Geometry: final body of the model. Coordinates: model frame, mm. A direction names the side the tool comes from. Give positions to 0.01 mm unless a question says otherwise; leave off trailing zeros. Write each loop counter-clockwise with the first axis right and the second up, starting at its lowest first coordinate (ties: lowest second). Pieces come first, ordered by that corner, then holes.
Q1. Reachability of faces 1 (the face through (28, 1, -50)), 2 (the face through (-12, 44, 31)), 3 (the face through (8, -1, -62.5)), 4 (the face through (-14, -22, 1)) from +Z, -Z, +X, -X, +Y, -Y: full face, straight path, thin tool, end or side. Return the list, or none.
Q2. Cut plane D-D on z = -58. Return the cut outline in (x, y), plus the area to 3 significant figures.
Q3. Cut plane B-B on y = -5. Return the cut outline in (x, z).
Q4. Draft query along X for faces 5 (the face through (0.816, 63.72, -19.983)), 6 (the face through (-8, -27, 1)), 7 (the face through (20, -1, 1)), 8 (the face through (0, -44, 1)). Return one class per face: pulls with the +X half, pulls with the -X half, needs draft (parallel to the pull), parting line crosses it, or undercut.
Q5. Pin query (flat end, axial travel): pin 1 (12.5 mm diameter, centred on x = 13, z = 29, fed in from +Y); pin 2 (4 mm diameter, centred on x = 7, y = 42, fed in from -Z); pin 3 (13 mm diameter, centred on x = -13, z = 12, fed in from -Y); pin 4 (11 mm diameter, centred on y = -25, z = -1.5, fed in from +X). Return the tip coordinate at first contact, or that it passes through.
Q6. Cut plane A-A on z = -75. Return the cut outline in (x, y).
Q7. Line query: L1, parallel to Z at x = 17.5, y = -39; L2, parallel to Y at x = -7, z = 20.5; L3, parallel to X at y = 62, z = 0. Output: solid intervals per line, ascending.
Q8. Cut plane C-C on x = 0. Return the cut outline in (y, z), plus the area to 3 significant figures.
```python
from build123d import *

# Parameters (mm, degrees)
BASE_BLOCK_SKETCH_W         = 40
BASE_BLOCK_SKETCH_H         = 88
BASE_BLOCK_DEPTH            = 50
C_CHANNEL_CUT_DEPTH         = 112.067547015
SLOTTED_LUG_DEPTH           = 40
LUG_START                   = 16
LUG_RIM_DEPTH               = 16
BOSS_CYLINDER_SKETCH_18_R   = 20
BOSS_CYLINDER_SKETCH_18_R_2 = 9
BOSS_CYLINDER_18_DEPTH      = 40
BOSS_EXTENSION_DEPTH        = 40
BOSS_BORE_CUT_DEPTH         = 40
GUSSET_RIB_A_SKETCH_W       = 40
GUSSET_RIB_A_SKETCH_H       = 4
GUSSET_RIB_A_DEPTH          = 10
GUSSET_RIB_B_SKETCH_W       = 40
GUSSET_RIB_B_SKETCH_H       = 4
GUSSET_RIB_B_DEPTH          = 10


with BuildPart() as part:
    # Base Block Sketch → Base Block (new, symmetric)
    with BuildSketch(Plane.XY):
        Rectangle(BASE_BLOCK_SKETCH_W, BASE_BLOCK_SKETCH_H)
    extrude(amount=BASE_BLOCK_DEPTH, both=True)

    # C-Channel Cut Sketch → C-Channel Cut (cut, through all)
    with BuildSketch(Plane.XY.offset(50)):
        Polygon((-20, 22), (-8, 22), (-8, 32), (8, 32), (8, -32), (-8, -32), (-8, -22), (-20, -22), align=None)
    extrude(amount=-C_CHANNEL_CUT_DEPTH, mode=Mode.SUBTRACT)

    # Slotted Lug Sketch → Slotted Lug (add, through all)
    with BuildSketch(Plane(origin=(20, 0, 0), x_dir=(0, 0, -1), z_dir=(1, 0, 0))):
        with BuildLine():
            Line((100, -40), (100, 40))
            ThreePointArc((100, 40), (75, 65), (50, 40))
            Line((50, 40), (50, -40))
            ThreePointArc((50, -40), (75, -65), (100, -40))
        make_face()
        with BuildLine():
            Line((62.5, -40), (62.5, 40))
            ThreePointArc((62.5, 40), (75, 52.5), (87.5, 40))
            Line((87.5, 40), (87.5, -40))
            ThreePointArc((87.5, -40), (75, -52.5), (62.5, -40))
        make_face(mode=Mode.SUBTRACT)
    extrude(amount=-SLOTTED_LUG_DEPTH)

    # Lug Rim Sketch → Lug Rim (add)
    with BuildSketch(Plane(origin=(20, 0, 0), x_dir=(0, 0, -1), z_dir=(1, 0, 0)).offset(LUG_START)):
        with BuildLine():
            Line((50, 40), (50, -40))
            ThreePointArc((50, -40), (75, -65), (100, -40))
            Line((100, -40), (100, 40))
            ThreePointArc((100, 40), (75, 65), (50, 40))
        make_face()
        with BuildLine():
            ThreePointArc((62.5, 40), (75, 52.5), (87.5, 40))
            Line((87.5, 40), (87.5, -40))
            ThreePointArc((87.5, -40), (75, -52.5), (62.5, -40))
            Line((62.5, -40), (62.5, 40))
        make_face(mode=Mode.SUBTRACT)
    extrude(amount=-LUG_RIM_DEPTH)

    # Boss Cylinder Sketch Ø18 → Boss Cylinder Ø18 (add)
    with BuildSketch(Plane(origin=(0, 44, 0), x_dir=(1, 0, 0), z_dir=(0, 1, 0))):
        with Locations(Location((0, 0, 0), (0, 0, 180))):
            Circle(BOSS_CYLINDER_SKETCH_18_R)
        with Locations(Location((0, 0, 0), (0, 0, 270))):
            Circle(BOSS_CYLINDER_SKETCH_18_R_2, mode=Mode.SUBTRACT)
    extrude(amount=BOSS_CYLINDER_18_DEPTH)

    # Boss Extension Sketch → Boss Extension (add)
    with BuildSketch(Plane(origin=(0, 44, 0), x_dir=(1, 0, 0), z_dir=(0, 1, 0))):
        with BuildLine():
            Line((-4.5, -19.48717527), (-4.5, -50))
            Line((-4.5, -50), (4.5, -50))
            Line((4.5, -50), (4.5, -19.48717527))
            ThreePointArc((4.5, -19.48717527), (0, -20), (-4.5, -19.48717527))
        make_face()
    extrude(amount=BOSS_EXTENSION_DEPTH)

    # Boss Bore Sketch → Boss Bore Cut (cut)
    with BuildSketch(Plane.ZY.offset(4.5)):
        Polygon((19.48717527, 84), (50, 44), (50, 84), align=None)
    extrude(amount=-BOSS_BORE_CUT_DEPTH, mode=Mode.SUBTRACT)

    # Gusset Rib A Sketch → Gusset Rib A (add)
    with BuildSketch(Plane(origin=(0, 0, -50), x_dir=(-1, 0, 0), z_dir=(0, 0, -1))):
        with Locations((0, 42)):
            Rectangle(GUSSET_RIB_A_SKETCH_W, GUSSET_RIB_A_SKETCH_H)
    extrude(amount=GUSSET_RIB_A_DEPTH)

    # Gusset Rib B Sketch → Gusset Rib B (add)
    with BuildSketch(Plane(origin=(0, 0, -50), x_dir=(-1, 0, 0), z_dir=(0, 0, -1))):
        with Locations((0, -42)):
            Rectangle(GUSSET_RIB_B_SKETCH_W, GUSSET_RIB_B_SKETCH_H)
    extrude(amount=GUSSET_RIB_B_DEPTH)


solid = part.part
```
Data:
1. face 1: +Z, +X, +Y, -Y
1. face 2: +Z, -X, +Y
1. face 3: +X, -X
1. face 4: +Z, -X
2. outline: (-20, -58.33) - (36, -58.33) - (36, 58.33) - (-20, 58.33) - close
2. area: 6,530 mm2
3. outline: (-20, -100) - (36, -100) - (36, -87.5) - (-20, -87.5) - close; (-20, -62.5) - (36, -62.5) - (36, -50) - (20, -50) - (20, 50) - (8, 50) - (8, -50) - (-20, -50) - close
4. face 5: parting line crosses it
4. face 6: undercut
4. face 7: pulls with the +X half
4. face 8: needs draft
5. pin 1: stops at y = 44
5. pin 2: stops at z = -100
5. pin 3: stops at y = -44
5. pin 4: stops at x = 20
6. outline: (-20, -65) - (36, -65) - (36, -52.5) - (-20, -52.5) - close; (-20, 52.5) - (36, 52.5) - (36, 65) - (-20, 65) - close
7. L1: z = -100 to -87.5, -62.5 to 50
7. L2: y = -44 to -32, 32 to 44
7. L3: x = -20 to -9, 9 to 20
8. outline: (-44, -50.32) arc R25 ccw to (-40, -100) - (40, -100) arc R25 ccw to (44, -50.32) - (44, -20) - (84, -20) - (84, -9) - (44, -9) - (44, 9) - (84, 9) - (84, 19.49) - (44, 50) - (32, 50) - (32, -50) - (-32, -50) - (-32, 50) - (-44, 50) - close; hole (-40, -87.5) - (40, -87.5) arc R12.5 ccw to (40, -62.5) - (-40, -62.5) arc R12.5 ccw to start
8. area: 7,340 mm2
